from build123d import *

# Parameters (mm, degrees)
EXTRUDE_1_DEPTH     = 5
SKETCH_2_R          = 7.5
CUT_EXTRUDE_1_DEPTH = 642.268274593


with BuildPart() as part:
    # 草图1 → 凸台-拉伸1 (new body)
    with BuildSketch(Plane.XY):
        with BuildLine():
            Line((0, 40), (600, 40))
            ThreePointArc((600, 40), (640, 0), (600, -40))
            Line((600, -40), (0, -40))
            ThreePointArc((0, -40), (-40, 0), (0, 40))
        make_face()
    extrude(amount=EXTRUDE_1_DEPTH)

    # 草图2 → 切除-拉伸1 (cut, through all)
    with BuildSketch(Plane.XY.offset(5)):
        Circle(SKETCH_2_R)
        with Locations((600, 0)):
            Circle(SKETCH_2_R)
    extrude(amount=-CUT_EXTRUDE_1_DEPTH, mode=Mode.SUBTRACT)


solid = part.part
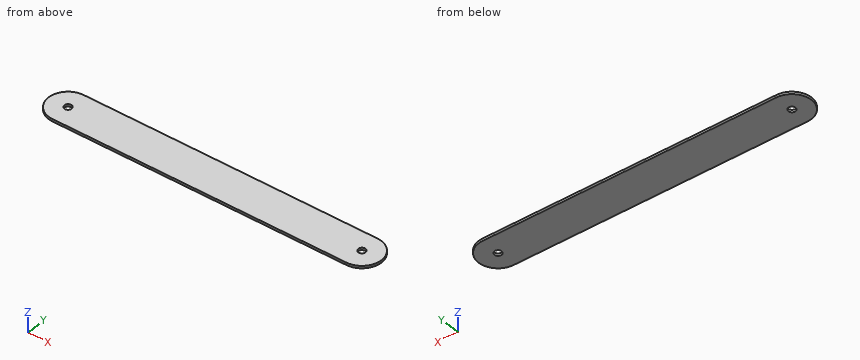
Read the model definition and answer for the solid it produces. Units are mm, in the model's axes. Give positions to 0.01 mm unless a question says otherwise; leave off trailing zeros. Write each loop counter-clockwise with the first axis right and the second up, starting at its lowest first coordinate (ties: lowest second). Pieces come first, ordered by that corner, then holes. Notation, with made-up numbers: (75.25, -29.5) -> (86.25, -29.5) arc R17 ccw to (86.25, -17.5) -> close; hole circle Ø8 at (71.25, 5). An arc over 180 degrees is marked (long way). Answer as a JSON object with one key per item and string values. Group by question number.
1) Consider L1, parallel to Y at x = 0, z = 3.7; L2, parallel to X at y = -24, z = 4.3; L3, parallel to X at y = -16.5, z = 4.6. Determine where each line is inside the solid, lowest interval first. Write a range as from..to.
2) Each of these flat-tipped pins is pushed along its axis until it touches: P1, Ø2, axis at y = 23, z = 1.5, coming from the -X side; P2, Ø12, axis at x = 600, y = 0, coming from the +Z side. Where does it stop, or does it pass through?
3) Find section A-A (y = 0). Write down the section's boundary in (x, z), and give its area (3 significant figures).
4) Find section C-C (y = -33). Write down the section's boundary in (x, z), and give its area (3 significant figures).
5) Find section B-B (z = 2.25). Write down the section's boundary in (x, y).
Values follow:
{
 "1": {"L1": "y = -40..-7.5, 7.5..40", "L2": "x = -32..632", "L3": "x = -36.44..636.44"},
 "2": {"P1": "stops at x = -33.41", "P2": "passes through"},
 "3": {"outline": "(-40, 0) -> (-7.5, 0) -> (-7.5, 5) -> (-40, 5) -> close; (7.5, 0) -> (592.5, 0) -> (592.5, 5) -> (7.5, 5) -> close; (607.5, 0) -> (640, 0) -> (640, 5) -> (607.5, 5) -> close", "area": "3,250 mm2"},
 "4": {"outline": "(-22.61, 0) -> (622.61, 0) -> (622.61, 5) -> (-22.61, 5) -> close", "area": "3,230 mm2"},
 "5": {"outline": "(0, -40) -> (600, -40) arc R40 ccw to (600, 40) -> (0, 40) arc R40 ccw to start; hole circle Ø15 at (0, 0); hole circle Ø15 at (600, 0)"}
}
